Check sheet for the modelled part. Datum: model origin and axes. Units: mm. Round coordinates to 2 decimals unless told otherwise and drop trailing zeros. Loops run counter-clockwise (first coordinate to the right, second up) from the corner with the lowest first, then second, coordinate; pieces in that order, holes last. Notation, with made-up numbers: (2.5, 1.5) - (29.5, 1.5) arc R14 cw to (29.5, 28.5) - close; hole circle Ø3 at (62, 55). An arc over 180 degrees is marked (long way). Put each result on its own line as item: value.
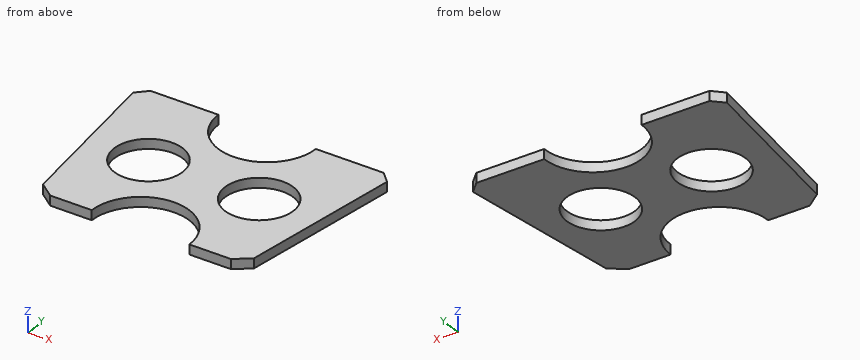
```python
from build123d import *

# Parameters (mm, degrees)
SKETCH1_R           = 35
BOSS_EXTRUDE1_DEPTH = 10


with BuildPart() as part:
    # Sketch1 → Boss-Extrude1 (new body)
    with BuildSketch(Plane.XY):
        with BuildLine():
            Line((50, 95), (119.5, 95))
            Line((119.5, 95), (130.104651163, 84.395348837))
            Line((130.104651163, 84.395348837), (108.065454151, -83.102548453))
            Line((108.065454151, -83.102548453), (92.562714257, -95))
            Line((92.562714257, -95), (50, -95))
            ThreePointArc((50, -95), (0, -45), (-50, -95))
            Line((-50, -95), (-92.562714257, -95))
            Line((-92.562714257, -95), (-108.065454151, -83.102548453))
            Line((-108.065454151, -83.102548453), (-130.104651163, 84.395348837))
            Line((-130.104651163, 84.395348837), (-119.5, 95))
            Line((-119.5, 95), (-50, 95))
            ThreePointArc((-50, 95), (0, 45), (50, 95))
        make_face()
        with Locations((56.75, 0)):
            Circle(SKETCH1_R, mode=Mode.SUBTRACT)
        with Locations(Location((-56.75, 0, 0), (0, 0, 180))):
            Circle(SKETCH1_R, mode=Mode.SUBTRACT)
    extrude(amount=BOSS_EXTRUDE1_DEPTH)


solid = part.part
```
Item 1: Section check A-A on x = 56.75. Enter the section's corners in (y, z).
Filled sheet:
outline: (-95, 0) - (-35, 0) - (-35, 10) - (-95, 10) - close; (35, 0) - (95, 0) - (95, 10) - (35, 10) - close
Item 2: Thickness scan on line 1 (Y direction, x = 56.75, z = 5); line 2 (Y direction, x = 46, z = 4.5); line 3 (X direction, y = -62, z = 7.5). Record the ranges inside material, lowest first. Write a range as from..to.
Filled sheet:
line 1: -95..-35, 35..95
line 2: -75.4..-33.31, 33.31..75.4
line 3: -110.84..-37.56, 37.56..110.84
Item 3: Section check D-D on y = 80. Enter the section's corners in (x, z).
Filled sheet:
outline: (-129.53, 0) - (-47.7, 0) - (-47.7, 10) - (-129.53, 10) - close; (47.7, 0) - (129.53, 0) - (129.53, 10) - (47.7, 10) - close
Item 4: Section check B-B on y = 0. Enter the section's corners in (x, z), then the cut area to 3 significant figures.
Filled sheet:
outline: (-119, 0) - (-91.75, 0) - (-91.75, 10) - (-119, 10) - close; (-21.75, 0) - (21.75, 0) - (21.75, 10) - (-21.75, 10) - close; (91.75, 0) - (119, 0) - (119, 10) - (91.75, 10) - close
area: 980 mm²
Item 5: Go/stop test with flat-tipped pins: pin 1 (4 mm diameter, centred on x = -91, y = 4, fed in from -Z); pin 2 (1.5 mm diameter, centred on x = -6.5, z = 5.5, fed in from -Y); pin 3 (1 mm diameter, centred on x = -1.5, z = 5, fed in from +Y). Record where each tip stops, or that it passes through.
Filled sheet:
pin 1: z = 0
pin 2: y = -45.53
pin 3: y = 45.04
Item 6: Section check C-C on z = 8. Enter the section's corners in (x, y).
Filled sheet:
outline: (-130.1, 84.4) - (-108.07, -83.1) - (-92.56, -95) - (-50, -95) arc R50 cw to (50, -95) - (92.56, -95) - (108.07, -83.1) - (130.1, 84.4) - (119.5, 95) - (50, 95) arc R50 cw to (-50, 95) - (-119.5, 95) - close; hole circle Ø70 at (-56.75, 0); hole circle Ø70 at (56.75, 0)
